```python
from build123d import *

# Parameters (mm, degrees)
BOSS_EXTRUDE1_DEPTH  = 40
FILLET1_R            = 20
FILLET2_R            = 5
BOSS_EXTRUDE2_DEPTH  = 10
FILLET3_R            = 5
FILLET4_R            = 2
BOSS_EXTRUDE6_DEPTH  = 100
BOSS_EXTRUDE8_DEPTH  = 4
CUT_EXTRUDE5_DEPTH   = 102
BOSS_EXTRUDE14_DEPTH = 30
CUT_EXTRUDE4_DEPTH   = 100
SKETCH25_W           = 2
SKETCH25_H           = 22.692372085
SKETCH25_H_2         = 22.697350811
BOSS_EXTRUDE15_DEPTH = 30
SKETCH26_R           = 10
BOSS_EXTRUDE16_DEPTH = 26.073999752
FILLET5_R            = 5


with BuildPart() as part:
    # Sketch2 → Boss-Extrude1 (new body)
    with BuildSketch(Plane(origin=(0, 0, 0), x_dir=(0, 0, -1), z_dir=(1, 0, 0))):
        Polygon((0, 0), (0, 50), (50, 50), (50, 29.410176709), (65.452441178, 21.589257338), (58.276483048, 0.061382948), (53.5278156, 0.061382948), (50, 9.231987855), (50, 0), align=None)
    extrude(amount=BOSS_EXTRUDE1_DEPTH)

    # Fillet1
    fillet1_edges = [part.edges().sort_by_distance(p)[0] for p in [
        (20, 50, 0),
    ]]
    fillet(fillet1_edges, radius=FILLET1_R)

    # Fillet2
    fillet2_edges = [part.edges().sort_by_distance(p)[0] for p in [
        (20, 0, 0),
    ]]
    fillet(fillet2_edges, radius=FILLET2_R)

    # Sketch4 → Boss-Extrude2 (add, symmetric)
    with BuildSketch(Plane(origin=(20, 0, 0), x_dir=(0, 0, -1), z_dir=(1, 0, 0))):
        Polygon((15, 0), (11.097402588, -30.529005874), (31.097402588, -30.529005874), (35, 0), align=None)
    extrude(amount=BOSS_EXTRUDE2_DEPTH, both=True)

    # Sketch5 → Revolve1 (revolve)
    with BuildSketch(Plane(origin=(20, 0, 0), x_dir=(0, 0, -1), z_dir=(1, 0, 0)), mode=Mode.PRIVATE) as revolve1_sk:
        Polygon((21.097402588, -30.529005874), (27.664898482, -30.529005874), (21.097402588, -65.678202337), align=None)
    revolve(revolve1_sk.sketch.rotate(Axis((20, -30.529005874, -21.097402588), (0, -1, 0)), 180), axis=Axis((20, -30.529005874, -21.097402588), (0, -1, 0)))

    # Fillet3
    fillet3_edges = [part.edges().sort_by_distance(p)[0] for p in [
        (20, 0.061382948, -53.5278156),
    ]]
    fillet(fillet3_edges, radius=FILLET3_R)

    # Fillet4
    fillet4_edges = [part.edges().sort_by_distance(p)[0] for p in [
        (20, 50, -50),
    ]]
    fillet(fillet4_edges, radius=FILLET4_R)

    # Sketch7 → Boss-Extrude6 (add)
    with BuildSketch(Plane(origin=(0, -17.47680662, -52.430419859), x_dir=(-1, 0, 0), z_dir=(0, -0.3162277660168374, -0.9486832980505141))):
        Polygon((-5.963000124, 18.486875023), (-16, 8.348197136), (-24, 8.348197136), (-34.036999876, 18.486875023), (-34.036999876, 46.955249244), (-5.963000124, 46.955249244), align=None)
    extrude(amount=BOSS_EXTRUDE6_DEPTH)

    # Sketch10 → Boss-Extrude8 (add, symmetric)
    with BuildSketch(Plane(origin=(20, 0, 0), x_dir=(0, 0, -1), z_dir=(1, 0, 0))):
        Polygon((147.227393234, -40.276025309), (132.358652474, -35.319778389), (134.836775442, -50.433902239), align=None)
        Polygon((132.358652474, -35.319778389), (117.489911715, -30.363531469), (119.968034683, -45.477655319), align=None)
        Polygon((117.489911715, -30.363531469), (101.885021683, -25.161901459), (104.363144652, -40.276025309), align=None)
        Polygon((101.885021683, -25.161901459), (86.280131652, -19.960271448), (88.75825462, -35.074395299), align=None)
        Polygon((86.280131652, -19.960271448), (70.675241621, -14.758641438), (73.153364589, -29.872765288), align=None)
        Polygon((70.675241621, -14.758641438), (55.07035159, -9.557011428), (57.548474558, -24.671135278), align=None)
    extrude(amount=BOSS_EXTRUDE8_DEPTH, both=True)

    # Sketch23 → Cut-Extrude5 (cut)
    with BuildSketch(Plane(origin=(0, -49.099583221, -147.298749664), x_dir=(-1, 0, 0), z_dir=(0, -0.3162277660168373, -0.948683298050514))):
        Polygon((-16, -5.206668435), (-16, 8.348197136), (-20, -5.214113496), align=None)
        Polygon((-24, -5.206668435), (-24, 8.348197136), (-20, -5.214113496), align=None)
    extrude(amount=-CUT_EXTRUDE5_DEPTH, mode=Mode.SUBTRACT)

    # Sketch24 → Boss-Extrude14 (add)
    with BuildSketch(Plane(origin=(0, -49.099583221, -147.298749664), x_dir=(-1, 0, 0), z_dir=(0, -0.3162277660168373, -0.948683298050514))):
        Polygon((-5.963000124, 18.486875023), (-5.963000124, 46.955249244), (-34.036999876, 46.955249244), (-34.036999876, 18.486875023), (-24, 8.348197136), (-16, 8.348197136), align=None)
    extrude(amount=BOSS_EXTRUDE14_DEPTH)

    # Sketch20 → Cut-Extrude4 (cut, symmetric)
    with BuildSketch(Plane(origin=(0, -49.099583221, -147.298749664), x_dir=(-1, 0, 0), z_dir=(0, -0.3162277660168373, -0.948683298050514))):
        Polygon((-34.036999876, 41.184225834), (-30.780503979, 46.955249244), (-34.036999876, 46.955249244), align=None)
        Polygon((-5.963000124, 41.184225834), (-9.219496021, 46.955249244), (-5.963000124, 46.955249244), align=None)
    extrude(amount=CUT_EXTRUDE4_DEPTH, both=True, mode=Mode.SUBTRACT)

    # Sketch25 → Boss-Extrude15 (add)
    with BuildSketch(Plane(origin=(0, -58.586416202, -175.759248606), x_dir=(-1, 0, 0), z_dir=(0, -0.31622776601683655, -0.9486832980505142))):
        with Locations((-33.036999876, 29.833061066)):
            Rectangle(SKETCH25_W, SKETCH25_H)
        with Locations((-6.963000124, 29.835550428)):
            Rectangle(SKETCH25_W, SKETCH25_H_2)
    extrude(amount=BOSS_EXTRUDE15_DEPTH)

    # Sketch26 → Boss-Extrude16 (add)
    with BuildSketch(Plane(origin=(34.036999876, 0, 0), x_dir=(0, 0, -1), z_dir=(1, 0, 0))):
        with Locations((200.721074436, -35.457593279)):
            Circle(SKETCH26_R)
    extrude(amount=-BOSS_EXTRUDE16_DEPTH)

    # Fillet5
    fillet5_edges = [part.edges().sort_by_distance(p)[0] for p in [
        (33.036999876, -50.535059615, -210.065810737),
        (33.036999876, -29.007185225, -217.241768866),
        (6.963000124, -29.00246199, -217.243343278),
        (6.963000124, -50.535059615, -210.065810737),
    ]]
    fillet(fillet5_edges, radius=FILLET5_R)

    # Sketch28 → Revolve3 (revolve)
    with BuildSketch(Plane(origin=(20, 0, 0), x_dir=(0, 0, -1), z_dir=(1, 0, 0))):
        Polygon((50, 33.769630528), (50, 39.271662622), (262.981733141, 137.079749362), (265.068381635, 132.535973612), align=None)
    revolve(axis=Axis((20, 39.271662622, -50), (0, 0.4173296987488473, -0.9087551499398484)))


solid = part.part
```
Here's how the part is built. I have some questions about the finished solid (model axes, mm). A direction names the side the tool comes from. Give positions to 0.01 mm unless a question says otherwise; leave off trailing zeros. Use CSV: the item, a comma, the result in double quotes. Start each with the question number.
Item 1: On a 3-axis mill with a long thin cutter (end or side, diameter ignored), from which of +Z, -Z, +X, -X, +Y, -Y can I reach the whole of each face in a straight line? I mean faces 1 (the flat face through (17.083, -15.676, -61.821)), 2 (the flat face through (20.056, -36.135, -118.436)), 3 (the flat face through (7.963, -32, -190)). Say none if no direction works.
Item 2: I'm going to push flat-ended pins straight in: P1, Ø12, axis at y = -19, z = -27.5, coming from the +X side; P2, Ø6, axis at x = 26.5, y = -41.5, coming from the -Z side; P3, Ø6, axis at x = 17, y = 58.5, coming from the +Z side. Where does each tip first touch, or does it pass through?
Item 3: If I drill on probe 1 along X at (y, z) = (-29.5, -27.5); probe 2 along Y at (x, z) = (23.5, -42); probe 3 along X at (y, z) = (20.5, -69), over which ranges is the centre line in solid material (lowest first)? Write a range as [from, to].
Item 4: Thinking about a two-plate mould opening in Z: for faces 4 (the flat face through (10, -15, -23)), 5 (the flat face through (7.6, 3.5, -128.9)), 6 (the flat face through (20.14, -15.48, -33.02)), which applies, pulls with the +Z half, pulls with the -Z half, needs draft (parallel to the pull), parting line crosses it, or undercut?
Answer block:
1,face 1,"-X, -Y"
1,face 2,"+X, -X, -Y"
1,face 3,"none"
2,P1,"stops at x = 30"
2,P2,"stops at z = -210.25"
2,P3,"stops at z = -74.71"
3,probe 1,"x = [10, 30]"
3,probe 2,"y = [0, 50]"
3,probe 3,"x = [6.01, 33.99]"
4,face 4,"needs draft"
4,face 5,"pulls with the -Z half"
4,face 6,"undercut"
